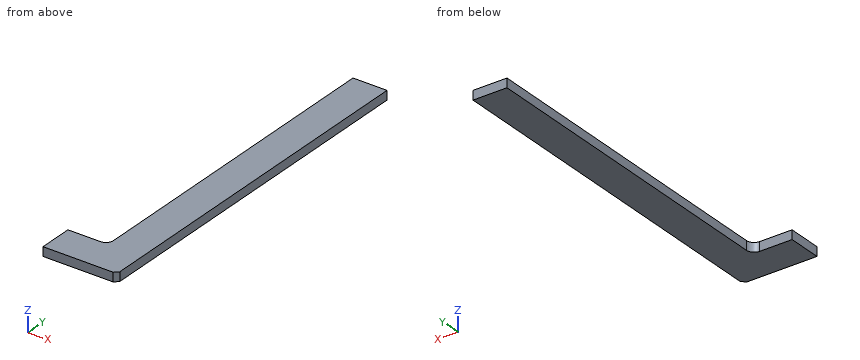
from build123d import *

# Parameters (mm, degrees)
SKETCH_1_W          = 98
SKETCH_1_H          = 488
EXTRUDE_1_DEPTH     = 6
CUT_EXTRUDE_1_REACH = 251.161
SKETCH_2_W          = 53
SKETCH_2_H          = 443
FILLET_1_R          = 10
CHAMFER_1_SIZE      = 5


with BuildPart() as part:
    # 草图1 → 凸台-拉伸1 (new, symmetric)
    with BuildSketch(Plane.XY):
        Rectangle(SKETCH_1_W, SKETCH_1_H)
    extrude(amount=EXTRUDE_1_DEPTH, both=True)

    # 草图2 → 切除-拉伸1 (cut, up to next)
    with BuildSketch(Plane.XY.offset(6), mode=Mode.PRIVATE) as cut_extrude_1_sk1:
        with Locations((-22.5, 22.5)):
            Rectangle(SKETCH_2_W, SKETCH_2_H)
    cut_extrude_1_tool1 = extrude(cut_extrude_1_sk1.sketch, amount=-CUT_EXTRUDE_1_REACH, mode=Mode.PRIVATE) & part.part
    add(cut_extrude_1_tool1.solids().sort_by_distance((-22.5, 22.5, 6))[0], mode=Mode.SUBTRACT)

    # 圆角1
    fillet_1_edges = [part.edges().sort_by_distance(p)[0] for p in [
        (4, -199, 0),
    ]]
    fillet(fillet_1_edges, radius=FILLET_1_R)

    # 倒角1
    chamfer_1_edges = [part.edges().sort_by_distance(p)[0] for p in [
        (49, -244, 0),
    ]]
    chamfer(chamfer_1_edges, length=CHAMFER_1_SIZE)


solid = part.part
The listing builds one solid part. Answer for the finished solid, in the listing's coordinates (mm). Coordinates: 2 decimals unless noted, no trailing zeros. Write each loop counter-clockwise with the first axis right and the second up, starting at its lowest first coordinate (ties: lowest second). Pieces come first, ordered by that corner, then holes. Notation, with made-up numbers: (46.5, -5.75) - (105.5, -5.75) arc R20 cw to (105.5, 15.25) - close; hole circle Ø4 at (70.5, 71). An arc over 180 degrees is marked (long way). Return JSON: item names as keys, results as strings.
1. This flat-tipped pin is pushed along its axis until it touches: pin 1 Ø6 at (y, z) = (67, 3) entering from -X. Where does it stop, or does it pass through?
Final values:
{"pin 1": "x = 4"}
2. Consider line 1 along X through (y, z) = (-66.5, -1.75); line 2 along Y through (x, z) = (-10, 5). Determine where each line is inside the solid, lowest interval first.
Final values:
{"line 1": "4 to 49", "line 2": "-244 to -199"}
3. The part is cut by section A-A on z = -1. Determine the outline of the cut face in (x, y).
Final values:
{"outline": "(-49, -244) - (44, -244) - (49, -239) - (49, 244) - (4, 244) - (4, -189) arc R10 cw to (-6, -199) - (-49, -199) - close"}
4. The part is cut by section C-C on y = 28.5. Determine the outline of the cut face in (x, z).
Final values:
{"outline": "(4, -6) - (49, -6) - (49, 6) - (4, 6) - close"}
5. The part is cut by section B-B on x = -30. Determine the outline of the cut face in (y, z), then the cut area to 3 significant figures.
Final values:
{"outline": "(-244, -6) - (-199, -6) - (-199, 6) - (-244, 6) - close", "area": "540 mm^2"}
